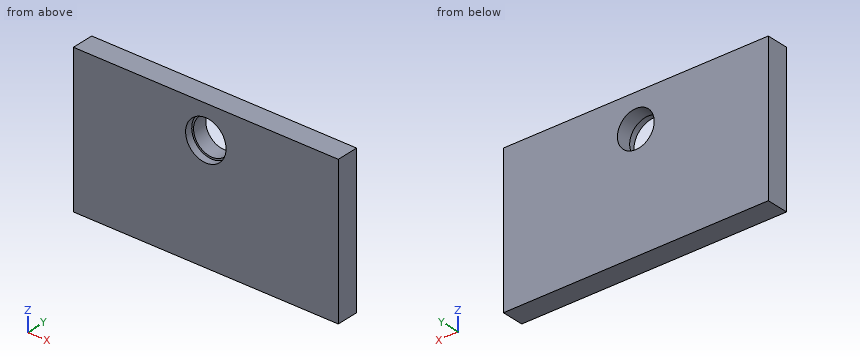
from build123d import *

# Parameters (mm, degrees)
SKETCH_1_W          = 360
SKETCH_1_H          = 200
EXTRUDE_1_DEPTH     = 30
SKETCH_2_R          = 25
CUT_EXTRUDE_1_DEPTH = 209.086520467
SKETCH_3_R          = 27.5
CUT_EXTRUDE_2_DEPTH = 10


with BuildPart() as part:
    # 草图1 → 凸台-拉伸1 (new body)
    with BuildSketch(Plane(origin=(0, 0, 0), x_dir=(1, 0, 0), z_dir=(0, 1, 0))):
        Rectangle(SKETCH_1_W, SKETCH_1_H)
    extrude(amount=EXTRUDE_1_DEPTH)

    # 草图2 → 切除-拉伸1 (cut, through all)
    with BuildSketch(Plane.XZ):
        with Locations(Location((0, 55, 0), (0, 0, 270))):
            Circle(SKETCH_2_R)
    extrude(amount=-CUT_EXTRUDE_1_DEPTH, mode=Mode.SUBTRACT)

    # 草图3 → 切除-拉伸2 (cut)
    with BuildSketch(Plane.XZ):
        with Locations(Location((0, 55, 0), (0, 0, 270))):
            Circle(SKETCH_3_R)
    extrude(amount=-CUT_EXTRUDE_2_DEPTH, mode=Mode.SUBTRACT)


solid = part.part
For this review, take the finished solid that the model builds, in its own axes (mm). Coordinates: 2 decimals unless noted, no trailing zeros. Write each loop counter-clockwise with the first axis right and the second up, starting at its lowest first coordinate (ties: lowest second). Pieces come first, ordered by that corner, then holes. Notation, with made-up numbers: (83.25, -10) -> (116.25, -10) arc R12 ccw to (116.25, 8) -> close; hole circle Ø4 at (-5, -27). An arc over 180 degrees is marked (long way). Write each question's results on one line, items separated by ' | '. Start each with the question number.
1) Insertion check: pin 1 (5 mm diameter, centred on x = -69.5, z = -15, fed in from -Y). The pin has a flat end and moves straight along its axis. Give the tip position at first contact, or say it passes through.
2) Consider section A-A (z = 55). Write out the cut boundary in (x, y), plus the area to 3 significant figures.
3) Consider section C-C (y = 16). Write out the cut boundary in (x, z).
4) Wall thickness on L1, parallel to X at y = 25.75, z = 55; L2, parallel to X at y = 5.75, z = 55: over which ranges is each line inside the solid? List them lowest first. Write a range as [from, to].
5) Consider section B-B (x = 0). Write out the cut boundary in (y, z).
Geometry says:
1) pin 1: y = 0
2) outline: (-180, 0) -> (-27.5, 0) -> (-27.5, 10) -> (-25, 10) -> (-25, 30) -> (-180, 30) -> close; (25, 10) -> (27.5, 10) -> (27.5, 0) -> (180, 0) -> (180, 30) -> (25, 30) -> close | area: 9,250 mm^2
3) outline: (-180, -100) -> (180, -100) -> (180, 100) -> (-180, 100) -> close; hole circle Ø50 at (0, 55)
4) L1: [-180, -25], [25, 180] | L2: [-180, -27.5], [27.5, 180]
5) outline: (0, -100) -> (30, -100) -> (30, 30) -> (10, 30) -> (10, 27.5) -> (0, 27.5) -> close; (0, 82.5) -> (10, 82.5) -> (10, 80) -> (30, 80) -> (30, 100) -> (0, 100) -> close
